from build123d import *

# Parameters (mm, degrees)
BASE_BLOCK_SKETCH_W         = 166
BASE_BLOCK_SKETCH_H         = 88
BASE_BLOCK_166X88X32_DEPTH  = 32
BORED_BOSS_SKETCH_R         = 44
BORED_BOSS_SKETCH_R_2       = 12.5
BORED_BOSS_88_BORE_25_DEPTH = 56
LUG_SKETCH_R                = 16
PIERCED_LUG_DEPTH           = 28


with BuildPart() as part:
    # Base Block Sketch → Base Block 166x88x32 (new body)
    with BuildSketch(Plane.XY):
        Rectangle(BASE_BLOCK_SKETCH_W, BASE_BLOCK_SKETCH_H)
    extrude(amount=BASE_BLOCK_166X88X32_DEPTH)

    # Bored Boss Sketch → Bored Boss Ø88 Bore Ø25 (add)
    with BuildSketch(Plane.XY.offset(32)):
        with Locations(Location((0, 0, 0), (0, 0, 270))):
            Circle(BORED_BOSS_SKETCH_R)
        Circle(BORED_BOSS_SKETCH_R_2, mode=Mode.SUBTRACT)
    extrude(amount=BORED_BOSS_88_BORE_25_DEPTH)

    # Lug Sketch → Pierced Lug (add)
    with BuildSketch(Plane(origin=(83, 0, 0), x_dir=(0, 0, -1), z_dir=(1, 0, 0))):
        with BuildLine():
            Line((0, 44), (0, -44))
            Line((0, -44), (47.072324291, -37.659945915))
            ThreePointArc((47.072324291, -37.659945915), (79.914891169, 2.541855154), (42, 38))
            Line((42, 38), (0, 44))
        make_face()
        with Locations((42, 0)):
            Circle(LUG_SKETCH_R, mode=Mode.SUBTRACT)
    pierced_lug = extrude(amount=-PIERCED_LUG_DEPTH)

    # Lug Mirror: Pierced Lug across plane
    add(pierced_lug.mirror(Plane(origin=(0, 0, 0), x_dir=(0, 0, 1), z_dir=(1, 0, 0))))


solid = part.part
Work out the finished part from the listing and answer in its coordinate system (mm). A direction names the side the tool comes from. Give positions to 0.01 mm unless a question says otherwise; leave off trailing zeros. Order: outer loops, then holes, each group sorted by start corner. A loop starts at its lowest first (then second) coordinate and runs counter-clockwise, first axis right, second up. Notation, with made-up numbers: (-9.75, 63) - (10.25, 63) arc R23 ccw to (10.25, 98) - close; hole circle Ø9 at (26.25, 62). An arc over 180 degrees is marked (long way). Answer as CSV lines item,"result". Start each with the question number.
Q1. Given pin 1 Ø19 at (y, z) = (0, -42) entering from -X; pin 2 Ø6 at (x, y) = (30, -21) entering from -Z; pin 3 Ø12 at (y, z) = (-33.5, 59.5) entering from -X; pin 4 Ø7.5 at (x, y) = (-4, 0.5) entering from +Z, each flat-ended and moving along its own axis, determine where each tip first touches the part or whether it passes through.
Q2. The part is cut by section C-C (z = -5.5). Write down the section's boundary in (x, y).
Q3. The mould has two halves that part along Z. Classify faces 4 (the face through (69.196, 0.703, -26.015)), 5 (the face through (-69.196, 0.703, -26.015)), 6 (the face through (69.2, 1.74, -79.96)), 7 (the face through (-83, 1, -11)): +Z half, -Z half, draft (parallel to the pull), parting line (faces both ways), or undercut.
Q4. The part is cut by section D-D (x = 8). Write down the section's boundary in (y, z), then the cut area to 3 significant figures.
Q5. The part is cut by section A-A (y = 0). Write down the section's boundary in (x, z).
Q6. For faces 1 (the face through (-1, -44, 16)), 2 (the face through (-1, 1, 0)), 3 (the face through (11.923, 3.755, 59.608)), determine the directions among +Z, -Z, +X, -X, +Y, -Y from which every point of the face is accessible in a straight line to the end or side of a thin tool.
Q7. Find the intervals of material crossed by L1, parallel to X at y = 32, z = -13; L2, parallel to Z at x = -38.5, y = 24.5; L3, parallel to Z at x = 28, y = 7, in increasing order. Write a range as [from, to].
Q8. The part is cut by section B-B (x = -73). Write down the section's boundary in (y, z).
Check result:
1,pin 1,"passes through"
1,pin 2,"stops at z = 0"
1,pin 3,"stops at x = -34.35"
1,pin 4,"stops at z = 32"
2,outline,"(-83, -43.26) - (-55, -43.26) - (-55, 43.21) - (-83, 43.21) - close; (55, -43.26) - (83, -43.26) - (83, 43.21) - (55, 43.21) - close"
3,face 4,"undercut"
3,face 5,"undercut"
3,face 6,"-Z half"
3,face 7,"draft"
4,outline,"(-44, 0) - (44, 0) - (44, 32) - (43.27, 32) - (43.27, 88) - (9.6, 88) - (9.6, 32) - (-9.6, 32) - (-9.6, 88) - (-43.27, 88) - (-43.27, 32) - (-44, 32) - close"
4,area,"6,590 mm²"
5,outline,"(-83, -80) - (-55, -80) - (-55, -58) - (-83, -58) - close; (-83, -26) - (-55, -26) - (-55, 0) - (55, 0) - (55, -26) - (83, -26) - (83, 32) - (44, 32) - (44, 88) - (12.5, 88) - (12.5, 32) - (-12.5, 32) - (-12.5, 88) - (-44, 88) - (-44, 32) - (-83, 32) - close; (55, -80) - (83, -80) - (83, -58) - (55, -58) - close"
6,face 1,"+Z, -Z, +X, -X, -Y"
6,face 2,"-Z, +Y, -Y"
6,face 3,"+Z"
7,L1,"x = [-83, -55], [55, 83]"
7,L2,"z = [0, 32]"
7,L3,"z = [0, 88]"
8,outline,"(-44, 0) - (-37.66, -47.07) arc R38 ccw to (38, -42) - (44, 0) - (44, 32) - (-44, 32) - close; hole circle Ø32 at (0, -42)"
